The model under review builds one solid part; all positions refer to its coordinate system, in mm. A direction names the side the tool comes from. Coordinates: 2 decimals unless noted, no trailing zeros. Order: outer loops, then holes, each group sorted by start corner. A loop starts at its lowest first (then second) coordinate and runs counter-clockwise, first axis right, second up.
```python
from build123d import *

# Parameters (mm, degrees)
SKETCH1_W           = 34
SKETCH1_H           = 35
BOSS_EXTRUDE1_DEPTH = 12
SKETCH2_R           = 2.1
CUT_EXTRUDE1_DEPTH  = 28.189152249
SKETCH3_W           = 43.383687714
SKETCH3_H           = 21.18675689
CUT_EXTRUDE2_DEPTH  = 1
SKETCH4_W           = 50.621361837
SKETCH4_H           = 17.880513978
CUT_EXTRUDE3_DEPTH  = 0.5
CUT_EXTRUDE4_DEPTH  = 1
SKETCH6_R           = 4.25
CUT_EXTRUDE5_DEPTH  = 6.5
SKETCH7_W           = 35.621240015
SKETCH7_H           = 1
CUT_EXTRUDE6_DEPTH  = 7.5
SKETCH8_W           = 34
SKETCH8_H           = 1
CUT_EXTRUDE7_DEPTH  = 7.5
FILLET1_R           = 3


with BuildPart() as part:
    # Sketch1 → Boss-Extrude1 (new body)
    with BuildSketch(Plane.XY):
        Rectangle(SKETCH1_W, SKETCH1_H)
    extrude(amount=BOSS_EXTRUDE1_DEPTH)

    # Sketch2 → Cut-Extrude1 (cut, through all)
    with BuildSketch(Plane.XY.offset(12)):
        with Locations((-8, -9)):
            Circle(SKETCH2_R)
        with Locations((8, -9)):
            Circle(SKETCH2_R)
        with BuildLine():
            Line((-6, 11.3), (6, 11.3))
            ThreePointArc((6, 11.3), (9.3, 8), (6, 4.7))
            Line((6, 4.7), (-6, 4.7))
            ThreePointArc((-6, 4.7), (-9.3, 8), (-6, 11.3))
        make_face()
    extrude(amount=-CUT_EXTRUDE1_DEPTH, mode=Mode.SUBTRACT)

    # Sketch3 → Cut-Extrude2 (cut)
    with BuildSketch(Plane.XY.offset(12)):
        with Locations((1.327871271, -7.093378445)):
            Rectangle(SKETCH3_W, SKETCH3_H)
    extrude(amount=-CUT_EXTRUDE2_DEPTH, mode=Mode.SUBTRACT)

    # Sketch4 → Cut-Extrude3 (cut)
    with BuildSketch(Plane(origin=(0, 0, 0), x_dir=(-1, 0, 0), z_dir=(0, 0, -1))):
        with Locations((0.547748923, -13.440256989)):
            Rectangle(SKETCH4_W, SKETCH4_H)
    extrude(amount=-CUT_EXTRUDE3_DEPTH, mode=Mode.SUBTRACT)

    # Sketch5 → Cut-Extrude4 (cut)
    with BuildSketch(Plane(origin=(0, 0, 0), x_dir=(-1, 0, 0), z_dir=(0, 0, -1))):
        Polygon((-23.912611607, 2), (26.337975431, 2), (17, -4.5), (-17, -4.5), align=None)
    extrude(amount=-CUT_EXTRUDE4_DEPTH, mode=Mode.SUBTRACT)

    # Sketch6 → Cut-Extrude5 (cut)
    with BuildSketch(Plane.XY.offset(11)):
        with Locations((8, -9)):
            Circle(SKETCH6_R)
        with Locations((-8, -9)):
            Circle(SKETCH6_R)
    extrude(amount=-CUT_EXTRUDE5_DEPTH, mode=Mode.SUBTRACT)

    # Sketch7 → Cut-Extrude6 (cut)
    with BuildSketch(Plane(origin=(0, 0, 1), x_dir=(-1, 0, 0), z_dir=(0, 0, -1))):
        with Locations((-0.810620008, 1.5)):
            Rectangle(SKETCH7_W, SKETCH7_H)
    extrude(amount=-CUT_EXTRUDE6_DEPTH, mode=Mode.SUBTRACT)

    # Sketch8 → Cut-Extrude7 (cut)
    with BuildSketch(Plane.XY.offset(11)):
        with Locations((0, -1.5)):
            Rectangle(SKETCH8_W, SKETCH8_H)
    extrude(amount=-CUT_EXTRUDE7_DEPTH, mode=Mode.SUBTRACT)

    # Fillet1
    fillet1_edges = [part.edges().sort_by_distance(p)[0] for p in [
        (17, -17.5, 5.75),
        (-17, -17.5, 5.75),
        (-17, 17.5, 6),
        (17, 17.5, 6),
    ]]
    fillet(fillet1_edges, radius=FILLET1_R)


solid = part.part
```
(1) Draft analysis for pull direction X (two halves, no side actions). For faces 6 (the face through (17, 0, 6)), 7 (the face through (0, -2, 7)), 8 (the face through (-9.3, 7.9, 6.1)), state which applies: released by +X, released by -X, zero draft, split by the parting line, or undercut.
A:
face 6: released by +X
face 7: zero draft
face 8: undercut
(2) For pin 1 Ø5 at (x, y) = (8, -9) entering from -Z; pin 2 Ø12 at (x, y) = (0, -4.5) entering from +Z; pin 3 Ø4.5 at (x, y) = (-4.5, -1) entering from -Z, all flat-tipped, find the tip position at first contact; note any pin that passes through.
A:
pin 1: stops at z = 0.5
pin 2: stops at z = 11
pin 3: stops at z = 1
(3) We need section C-C, the plane x = -2. Write out the cut boundary in (y, z), and give its area (3 significant figures).
A:
outline: (-17.5, 0.5) - (-4.5, 0.5) - (-4.5, 1) - (1, 1) - (1, 8.5) - (2, 8.5) - (2, 0) - (4.7, 0) - (4.7, 12) - (3.5, 12) - (3.5, 11) - (-1, 11) - (-1, 3.5) - (-2, 3.5) - (-2, 11) - (-17.5, 11) - close; (11.3, 0) - (17.5, 0) - (17.5, 12) - (11.3, 12) - close
area: 292 mm2
(4) Wall thickness on probe 1 along Y at (x, z) = (-2, 1.5); probe 2 along Y at (x, z) = (12, 4); probe 3 along Y at (x, z) = (11.5, 6.75): over which ranges is each line inside the solid? List them lowest first.
A:
probe 1: y = -17.5 to 1, 2 to 4.7, 11.3 to 17.5
probe 2: y = -17.5 to -2, -1 to 1, 2 to 17.5
probe 3: y = -17.5 to -11.41, -6.59 to -2, -1 to 1, 2 to 17.5
(5) We need section B-B, the plane y = 8. Write out the cut boundary in (x, z), and give its area (3 significant figures).
A:
outline: (-17, 0) - (-9.3, 0) - (-9.3, 12) - (-17, 12) - close; (9.3, 0) - (17, 0) - (17, 12) - (9.3, 12) - close
area: 185 mm2
(6) We need section D-D, the plane z = 1.5. Write out the cut boundary in (x, y), and give its area (3 significant figures).
A:
outline: (-17, -14.5) arc R3 ccw to (-14, -17.5) - (14, -17.5) arc R3 ccw to (17, -14.5) - (17, 1) - (-17, 1) - close; (-17, 2) - (17, 2) - (17, 14.5) arc R3 ccw to (14, 17.5) - (-14, 17.5) arc R3 ccw to (-17, 14.5) - close; hole circle Ø4.2 at (-8, -9); hole (-6, 4.7) - (6, 4.7) arc R3.3 ccw to (6, 11.3) - (-6, 11.3) arc R3.3 ccw to start; hole circle Ø4.2 at (8, -9)
area: 1,010 mm2
(7) We need section A-A, the plane z = 6.5. Write out the cut boundary in (x, y), and give its area (3 significant figures).
A:
outline: (-17, -14.5) arc R3 ccw to (-14, -17.5) - (14, -17.5) arc R3 ccw to (17, -14.5) - (17, -2) - (-17, -2) - close; (-17, -1) - (17, -1) - (17, 1) - (-17, 1) - close; (-17, 2) - (17, 2) - (17, 14.5) arc R3 ccw to (14, 17.5) - (-14, 17.5) arc R3 ccw to (-17, 14.5) - close; hole circle Ø8.5 at (-8, -9); hole (-6, 4.7) - (6, 4.7) arc R3.3 ccw to (6, 11.3) - (-6, 11.3) arc R3.3 ccw to start; hole circle Ø8.5 at (8, -9)
area: 887 mm2
(8) Machinability: for faces 1 (the face through (0, -2, 1)), 2 (the face through (0, 12, 0)), 3 (the face through (0, -1, 7)), 4 (the face through (0, 4.7, 6)), 5 (the face through (16.1, 16.64, 6.08)), which of the approach directions +Z, -Z, +X, -X, +Y, -Y give a long, thin tool a straight path to every point of the face, cutting with its end or side? Answer none if there is none.
A:
face 1: -Z, +X, -X
face 2: -Z, +X, -X, +Y, -Y
face 3: +Z, +X, -X
face 4: +Z, -Z
face 5: +Z, -Z, +X, +Y
